CAD build for the part. Positions are in the model's coordinates, mm. Face numbers are marked on the shaded views. A direction names the side the tool comes from. Coordinates: 2 decimals unless noted, no trailing zeros. Order: outer loops, then holes, each group sorted by start corner. A loop starts at its lowest first (then second) coordinate and runs counter-clockwise, first axis right, second up. Notation, with made-up numbers: (30.5, -3.5) - (51.5, -3.5) arc R25 ccw to (51.5, 29.5) - close; hole circle Ø10 at (-3, -30). An arc over 180 degrees is marked (long way). Use one line per item in the form item = value.
```python
from build123d import *

# Parameters (mm, degrees)
PLATE_PROFILE_R           = 3
PLATE_PROFILE_R_2         = 12
BASE_PLATE_132X64X5_DEPTH = 5
HUB_PROFILE_R             = 16
HUB_PROFILE_R_2           = 12
HUB_BOSS_DEPTH            = 13
HUB_RIB_10MM_REACH        = 77.525
RIB_PROFILE_WALL_W        = 198.049660708
RIB_PROFILE_WALL_H        = 10
RIB_PATTERN_4X_COUNT      = 4


with BuildPart() as part:
    # Plate Profile → Base Plate 132x64x5 (new body)
    with BuildSketch(Plane.XY):
        with BuildLine():
            Line((-60, -32), (60, -32))
            ThreePointArc((60, -32), (64.242640687, -30.242640687), (66, -26))
            Line((66, -26), (66, 26))
            ThreePointArc((66, 26), (64.242640687, 30.242640687), (60, 32))
            Line((60, 32), (-60, 32))
            ThreePointArc((-60, 32), (-64.242640687, 30.242640687), (-66, 26))
            Line((-66, 26), (-66, -26))
            ThreePointArc((-66, -26), (-64.242640687, -30.242640687), (-60, -32))
        make_face()
        with Locations((-60, 26)):
            Circle(PLATE_PROFILE_R, mode=Mode.SUBTRACT)
        with Locations((60, 26)):
            Circle(PLATE_PROFILE_R, mode=Mode.SUBTRACT)
        with Locations((60, -26)):
            Circle(PLATE_PROFILE_R, mode=Mode.SUBTRACT)
        with Locations((-60, -26)):
            Circle(PLATE_PROFILE_R, mode=Mode.SUBTRACT)
        Circle(PLATE_PROFILE_R_2, mode=Mode.SUBTRACT)
    extrude(amount=BASE_PLATE_132X64X5_DEPTH)

    # Hub Profile → Hub Boss (add)
    with BuildSketch(Plane.XY.offset(5)):
        with Locations(Location((0, 0, 0), (0, 0, 180))):
            Circle(HUB_PROFILE_R)
        Circle(HUB_PROFILE_R_2, mode=Mode.SUBTRACT)
    extrude(amount=HUB_BOSS_DEPTH)

    # Rib Profile wall → Hub Rib 10mm (add, up to next)
    with BuildSketch(Plane(origin=(-15.131216519, -15.131216519, 11.047117627), x_dir=(-0.672498511963, -0.672498511963, -0.309016994381), z_dir=(-0.218508012229, -0.218508012229, 0.951056516293)), mode=Mode.PRIVATE) as hub_rib_10mm_sk1:
        Rectangle(RIB_PROFILE_WALL_W, RIB_PROFILE_WALL_H)
    hub_rib_10mm_tool1 = extrude(hub_rib_10mm_sk1.sketch, amount=-HUB_RIB_10MM_REACH, mode=Mode.PRIVATE) - part.part
    hub_rib_10mm = hub_rib_10mm_tool1.solids().sort_by_distance((-15.131216519, -15.131216519, 11.047117627))[0]
    add(hub_rib_10mm)

    # Rib Pattern 4x: Hub Rib 10mm ×4 about axis
    rib_pattern_4x_axis = Axis((0, 0, 0), (0, 0, 1))
    for i in range(1, RIB_PATTERN_4X_COUNT):
        add(hub_rib_10mm.rotate(rib_pattern_4x_axis, i * 360 / RIB_PATTERN_4X_COUNT))


solid = part.part
```
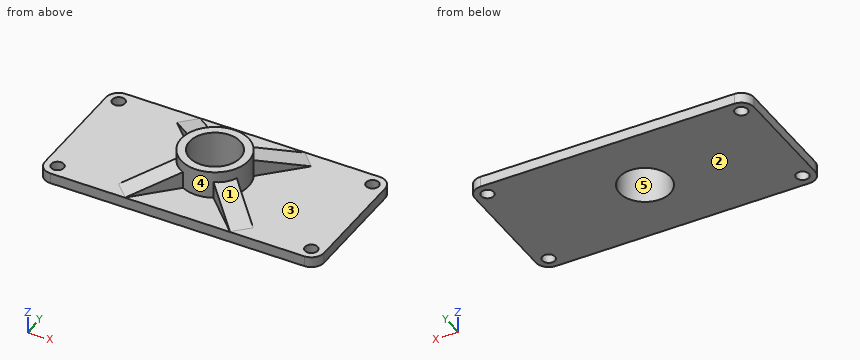
Item 1: Cut at C-C, the plane x = 0. Write the cut outline in (y, z), plus the area to 3 significant figures.
Derived:
outline = (-32, 0) - (-12, 0) - (-12, 18) - (-16, 18) - (-16, 5) - (-32, 5) - close; (12, 0) - (32, 0) - (32, 5) - (16, 5) - (16, 18) - (12, 18) - close
area = 304 mm²
Item 2: Drill centre lines: line 1 (Y direction, x = -60, z = 3.05); line 2 (Y direction, x = 0, z = 9.5); line 3 (Z direction, x = -37.5, y = 10.5). Where is each one in solid material? Low to high. Write a range as [from, to].
Derived:
line_1 = [-32, -29], [-23, 23], [29, 32]
line_2 = [-16, -12], [12, 16]
line_3 = [0, 5]
Item 3: Cut at B-B, the plane z = 3.25. Write the cut outline in (x, y).
Derived:
outline = (-66, -26) arc R6 ccw to (-60, -32) - (60, -32) arc R6 ccw to (66, -26) - (66, 26) arc R6 ccw to (60, 32) - (-60, 32) arc R6 ccw to (-66, 26) - close; hole circle Ø6 at (-60, -26); hole circle Ø6 at (-60, 26); hole circle Ø24 at (0, 0); hole circle Ø6 at (60, -26); hole circle Ø6 at (60, 26)
Item 4: 3-axis set-ups, long thin cutter, end or side, ignore diameter. For the marked faces 4 and 5: which of +Z, -Z, +X, -X, +Y, -Y reach the whole face in a straight line?
Derived:
face_4 = +Z
face_5 = +Z, -Z
Item 5: Cut at A-A, the plane y = 0. Write the cut outline in (x, z), plus the area to 3 significant figures.
Derived:
outline = (-66, 0) - (-12, 0) - (-12, 18) - (-16, 18) - (-16, 5) - (-66, 5) - close; (12, 0) - (66, 0) - (66, 5) - (16, 5) - (16, 18) - (12, 18) - close
area = 644 mm²
Item 6: Cut at D-D, the plane y = -9. Write the cut outline in (x, z).
Derived:
outline = (-66, 0) - (-7.94, 0) - (-7.94, 18) - (-13.23, 18) - (-13.23, 12.89) - (-16.07, 12.24) - (-16.07, 5) - (-66, 5) - close; (7.94, 0) - (66, 0) - (66, 5) - (16.07, 5) - (16.07, 12.24) - (13.23, 12.89) - (13.23, 18) - (7.94, 18) - close
Item 7: Drop flat-ended pins along their axis: pin 1 (19 mm diameter, centred on x = 0, y = 0, fed in from +Z); pin 2 (1.5 mm diameter, centred on x = 39.5, y = -19.5, fed in from +Z); pin 3 (3 mm diameter, centred on x = 7, z = 15.5, fed in from -Y) (3 decimals). Give the stop position or say it passes through.
Derived:
pin_1 = through
pin_2 = 5
pin_3 = -15.025
Item 8: Two-plate mould, pull along X, no slides. Class the marked faces 1, 2 and 3: +X half, -X half, draft (parallel to the pull), parting line (faces both ways), or undercut.
Derived:
face_1 = +X half
face_2 = draft
face_3 = undercut
